Job drawing, mm, ordinate dimensions from the low corner. One solid piece. A direction names the side the tool comes from. Round coordinates to 2 decimals unless told otherwise and drop trailing zeros. Order: outer loops, then holes, each group sorted by start corner. A loop starts at its lowest first (then second) coordinate and runs counter-clockwise, first axis right, second up. Notation, with made-up numbers: (6.5, -24) -> (46.5, -24) arc R20 cw to (46.5, 14) -> close; hole circle Ø10 at (54, 35.25). An arc over 180 degrees is marked (long way). Return JSON: item names as keys, results as strings. Group by question number.
Q1. Probe line 1 along Y through (x, z) = (1.7, 4.75); line 2 along X through (y, z) = (11, 4); line 3 along Z through (x, y) = (1.7, 5.5). List the from-to ranges inside material, lowest first.
Q2. Flat gauge pin, fed straight in: pin 1 (2 mm diameter, centred on y = 4.5, z = 1, fed in from -X). Where does the tip first touch, or does it go through?
Q3. Cut at C-C (y = 11.5). Write the cut outline in (x, z), then the cut area to 3 significant figures.
Q4. Which spindle directions (+Z, -Z, +X, -X, +Y, -Y) get a long thin tool onto all of the face, cutting with end or side? Do the marked faces 1 and 2. Say none if no direction does.
Q5. Cut at A-A (x = 2.5). Write the cut outline in (y, z).
Q6. Cut at B-B (z = 2.5). Write the cut outline in (x, y), then the cut area to 3 significant figures.
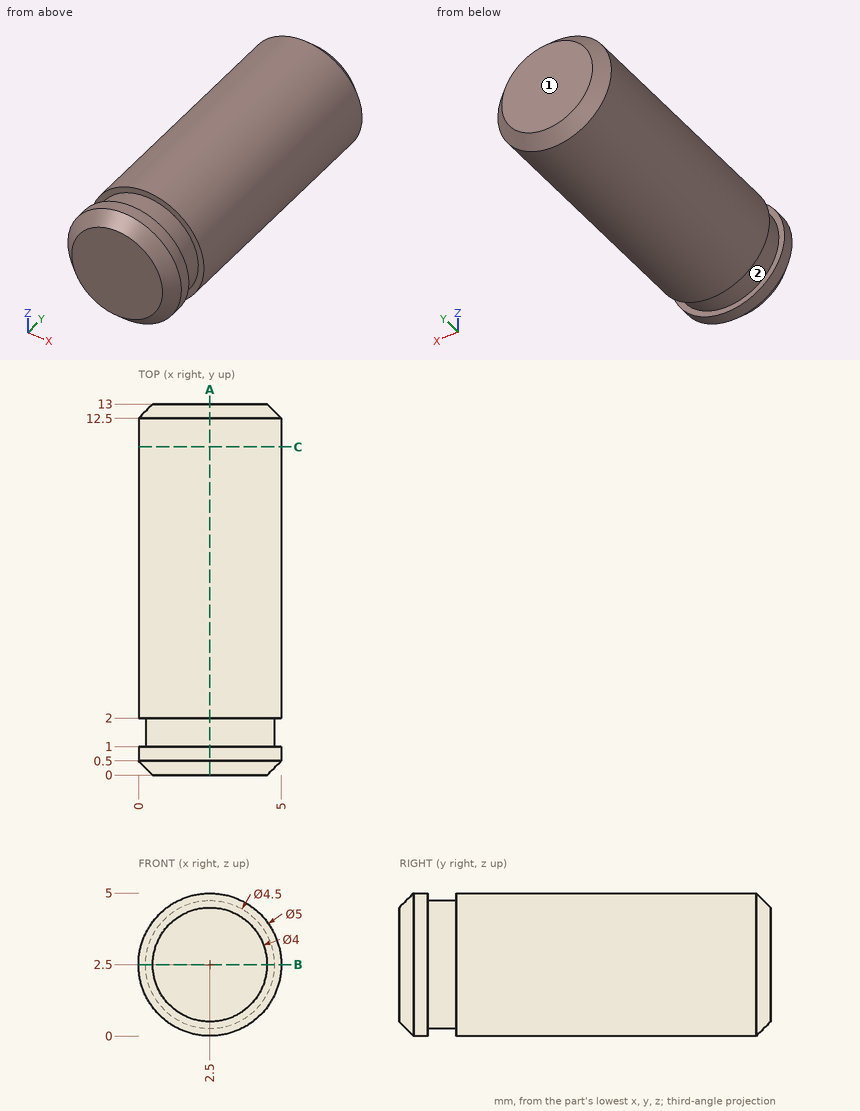
Solution:
{
 "1": {"line 1": "y = 0.39 to 1, 2 to 12.61", "line 2": "x = 0.5 to 4.5", "line 3": "z = 0.13 to 4.87"},
 "2": {"pin 1": "stops at x = 0.05"},
 "3": {"outline": "circle Ø5 at (2.5, 2.5)", "area": "19.6 mm²"},
 "4": {"face 1": "+Z, -Z, +X, -X, +Y", "face 2": "none"},
 "5": {"outline": "(0, 0.5) -> (0.5, 0) -> (1, 0) -> (1, 0.25) -> (2, 0.25) -> (2, 0) -> (12.5, 0) -> (13, 0.5) -> (13, 4.5) -> (12.5, 5) -> (2, 5) -> (2, 4.75) -> (1, 4.75) -> (1, 5) -> (0.5, 5) -> (0, 4.5) -> close"},
 "6": {"outline": "(0, 0.5) -> (0.5, 0) -> (4.5, 0) -> (5, 0.5) -> (5, 1) -> (4.75, 1) -> (4.75, 2) -> (5, 2) -> (5, 12.5) -> (4.5, 13) -> (0.5, 13) -> (0, 12.5) -> (0, 2) -> (0.25, 2) -> (0.25, 1) -> (0, 1) -> close", "area": "64.0 mm²"}
}
